Could you check a few things on this model? Use its own coordinates, in mm. Face numbers are marked on the shaded views. Round coordinates to 2 decimals unless told otherwise and drop trailing zeros. Write each loop counter-clockwise with the first axis right and the second up, starting at its lowest first coordinate (ties: lowest second). Pieces come first, ordered by that corner, then holes. Notation, with made-up numbers: (-22, 37) - (29, 37) arc R30 ccw to (29, 62) - close; hole circle Ø4 at (19.5, -9.5). An arc over 180 degrees is marked (long way). Put each result on its own line as item: value.
from build123d import *

# Parameters (mm, degrees)
SKETCH_1_W          = 39.5
SKETCH_1_H          = 26.7
EXTRUDE_1_DEPTH     = 41
EXTRUDE_2_DEPTH     = 4
SKETCH_3_W          = 2.15
SKETCH_3_H          = 4
CUT_EXTRUDE_1_DEPTH = 1.3


with BuildPart() as part:
    # 草图1 → 凸台-拉伸1 (new body)
    with BuildSketch(Plane(origin=(0, 0, 0), x_dir=(1, 0, 0), z_dir=(0, 1, 0))):
        with Locations((0, 13.35)):
            Rectangle(SKETCH_1_W, SKETCH_1_H)
    extrude(amount=EXTRUDE_1_DEPTH)

    # 草图2 → 凸台-拉伸2 (add)
    with BuildSketch(Plane(origin=(0, 0, 0), x_dir=(1, 0, 0), z_dir=(0, 1, 0))):
        with BuildLine():
            Line((-10, 0), (-5.217320496, -7.449562186))
            ThreePointArc((-5.217320496, -7.449562186), (0, -10.3), (5.217320496, -7.449562186))
            Line((5.217320496, -7.449562186), (10, 0))
            Line((10, 0), (-10, 0))
        make_face()
    extrude(amount=EXTRUDE_2_DEPTH)

    # 草图3 → 切除-旋转1 (revolve, cut)
    with BuildSketch(Plane.XY.offset(4.1), mode=Mode.PRIVATE) as cut_revolve_1_sk:
        with Locations((1.075, 2)):
            Rectangle(SKETCH_3_W, SKETCH_3_H)
    revolve(cut_revolve_1_sk.sketch.rotate(Axis((0, 0, 4.1), (0, 1, 0)), 270), axis=Axis((0, 0, 4.1), (0, 1, 0)), mode=Mode.SUBTRACT)

    # 草图4 → 旋转1 (revolve)
    with BuildSketch(Plane.XY.offset(4.1), mode=Mode.PRIVATE) as revolve_1_sk:
        with BuildLine():
            Line((0, 6.2), (1.6, 6.2))
            ThreePointArc((1.6, 6.2), (3.155634919, 5.555634919), (3.8, 4))
            Line((3.8, 4), (2, 4))
            Line((2, 4), (2, -5.5705))
            Line((2, -5.5705), (1.5705, -6))
            Line((1.5705, -6), (0, -6))
            Line((0, -6), (0, 6.2))
        make_face()
    revolve(revolve_1_sk.sketch.rotate(Axis((0, -6, 4.1), (0, 1, 0)), 270), axis=Axis((0, -6, 4.1), (0, 1, 0)))

    # 草图5 → 切除-拉伸1 (cut)
    with BuildSketch(Plane(origin=(0, 6.2, 0), x_dir=(1, 0, 0), z_dir=(0, 1, 0))):
        Polygon((-1.25, -3.378312164), (-1.25, -4.821687836), (0, -5.543375673), (1.25, -4.821687836), (1.25, -3.378312164), (0, -2.656624327), align=None)
    extrude(amount=-CUT_EXTRUDE_1_DEPTH, mode=Mode.SUBTRACT)


solid = part.part
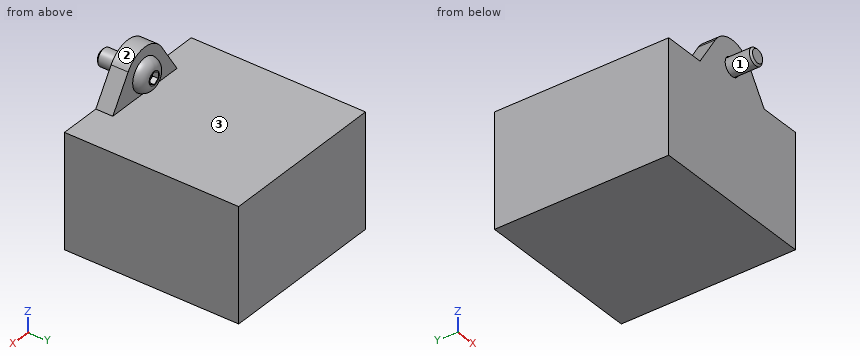
(1) I'm going to push flat-ended pins straight in: pin 1 (3.5 mm diameter, centred on x = 0, z = 4.1, fed in from +Y); pin 2 (12 mm diameter, centred on x = 1, y = 28.5, fed in from +Z); pin 3 (1 mm diameter, centred on y = 5.5, z = 4.5, fed in from +X). Where does each tip first touch, or does it pass through?
Values found:
pin 1: stops at y = 6.2
pin 2: stops at z = 0
pin 3: stops at x = 3.54
(2) If we mould it in two halves opening along X, with no side actions, what happens to the marked faces 1, 2 and 3? For each: pulls with the +X half, pulls with the -X half, needs draft (parallel to the pull), parting line crosses it, or undercut.
Values found:
face 1: undercut
face 2: parting line crosses it
face 3: needs draft
(3) Imagine slicing it at A-A, the plane y = 16.5. List the corners of the cut face in (x, z) for me, then the cut area to 3 significant figures.
Values found:
outline: (-19.75, -26.7) - (19.75, -26.7) - (19.75, 0) - (-19.75, 0) - close
area: 1,050 mm^2
(4) Imagine slicing it at D-D, the plane y = -1. List the corners of the cut face in (x, z) for me.
Values found:
outline: circle Ø4 at (0, 4.1)
(5) Imagine slicing it at B-B, the plane x = -6.5. List the corners of the cut face in (y, z) for me.
Values found:
outline: (0, -26.7) - (41, -26.7) - (41, 0) - (4, 0) - (4, 5.45) - (0, 5.45) - close
(6) Imagine slicing it at C-C, the plane z = -15. List the corners of the cut face in (x, y) for me, then the cut area to 3 significant figures.
Values found:
outline: (-19.75, 0) - (19.75, 0) - (19.75, 41) - (-19.75, 41) - close
area: 1,620 mm^2
(7) Please list where these lines run through material, in increasing order: probe 1 along Z at (x, y) = (-1, 0.5); probe 2 along X at (y, z) = (1, 4); probe 3 along Z at (x, y) = (-9.5, 17). Write a range as from..to.
Values found:
probe 1: z = -26.7..2.2, 2.37..5.83, 6..10.22
probe 2: x = -7.43..-2.15, -2..2, 2.15..7.43
probe 3: z = -26.7..0
